CAD build for the part. Positions are in the model's coordinates, mm. Face numbers are marked on the shaded views. A direction names the side the tool comes from. Coordinates: 2 decimals unless noted, no trailing zeros. Loops run counter-clockwise (first coordinate to the right, second up) from the corner with the lowest first, then second, coordinate; pieces in that order, holes last.
1) Which spindle directions (+Z, -Z, +X, -X, +Y, -Y) get a long thin tool onto all of the face, cutting with end or side? Do the marked faces 1, 2 and 3. Say none if no direction does.
2) Saw through at B-B, the plane y = -220. Write the cut outline in (x, z), and give its area (3 significant figures).
3) Wall check: line 1 along Z through (x, y) = (0, -230); line 2 along Z through (x, y) = (0, -156); line 3 along X through (y, z) = (-191.5, 10.5). Give the ranges that are in metal, low to high.
4) Saw through at A-A, the plane y = -186.5. Write the cut outline in (x, z).
5) Pin check, flat tips, straight feed: pin 1 Ø1.5 at (y, z) = (-218.5, 13.5) entering from +X; pin 2 Ø4 at (x, y) = (9, -199.5) entering from +Z; pin 3 Ø4 at (y, z) = (-264, -6) entering from -X. Stop position of each tip, or through.
6) Two-plate mould, pull along X, no slides. Class the marked faces 4, 5 and 6: +X half, -X half, draft (parallel to the pull), parting line (faces both ways), or undercut.
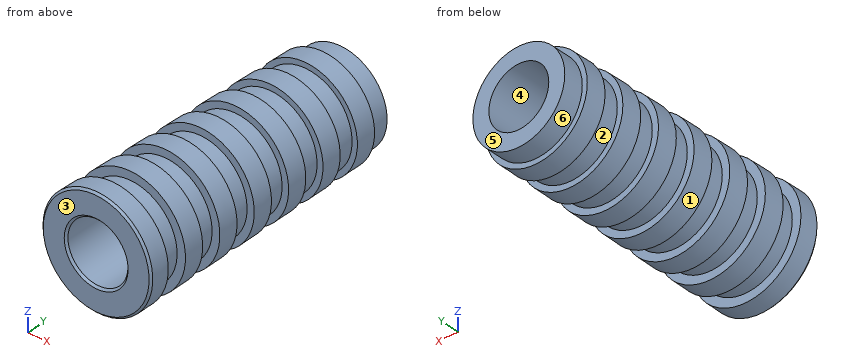
```python
from build123d import *


with BuildPart() as part:
    # 草图1 → 旋转1 (revolve)
    with BuildSketch(Plane(origin=(0, 0, 0), x_dir=(-1, 0, 0), z_dir=(0, 0, -1)), mode=Mode.PRIVATE) as revolve_1_sk:
        Polygon((-23, -215), (-26.422241501, -215), (-26.576207001, -225), (-23, -225), (-23, -235), (-26.730172501, -235), (-26.884138001, -245), (-23, -245), (-23, -255), (-27.038103501, -255), (-27.192069, -265), (-23, -265), (-23, -275), (-27.3460345, -275), (-27.484836909, -284.015163091), (-26.5, -285), (-16, -285), (-15, -284), (-15, -145), (-23, -145), (-23, -155), (-25.498448502, -155), (-25.652414002, -165), (-23, -165), (-23, -175), (-25.806379502, -175), (-25.960345002, -185), (-23, -185), (-23, -195), (-26.114310502, -195), (-26.268276001, -205), (-23, -205), align=None)
    revolve(revolve_1_sk.sketch.rotate(Axis((0, -285, 0), (0, 1, 0)), 180), axis=Axis((0, -285, 0), (0, 1, 0)))


solid = part.part
```
Data:
1. face 1: +Y
1. face 2: none
1. face 3: +Z, -Z, +X, -X, -Y
2. outline: circle Ø53 at (0, 0); hole circle Ø30 at (0, 0)
2. area: 1,500 mm2
3. line 1: z = -23 to -15, 15 to 23
3. line 2: z = -25.51 to -15, 15 to 25.51
3. line 3: x = -20.46 to -10.71, 10.71 to 20.46
4. outline: circle Ø46 at (0, 0); hole circle Ø30 at (0, 0)
5. pin 1: stops at x = 23.2
5. pin 2: stops at z = 25.23
5. pin 3: stops at x = -26.88
6. face 4: undercut
6. face 5: draft
6. face 6: parting line
